```python
from build123d import *

# Parameters (mm, degrees)
SKETCH1_W              = 100
SKETCH1_H              = 100
BOSS_EXTRUDE1_DEPTH    = 10
M12_TAPPED_HOLE1_D     = 10.2
M12_TAPPED_HOLE1_DEPTH = 29.25
M12_TAPPED_HOLE1_TIP   = 3.064389157


with BuildPart() as part:
    # Sketch1 → Boss-Extrude1 (new body)
    with BuildSketch(Plane.XY):
        Rectangle(SKETCH1_W, SKETCH1_H)
    extrude(amount=BOSS_EXTRUDE1_DEPTH)

    # M12 Tapped Hole1
    with Locations(Plane.XY.offset(10)):
        with Locations((0, 30), (0, -30)):
            Hole(M12_TAPPED_HOLE1_D / 2, depth=M12_TAPPED_HOLE1_DEPTH)
            with Locations((0, 0, -(M12_TAPPED_HOLE1_DEPTH + M12_TAPPED_HOLE1_TIP / 2))):  # 118° drill point
                Cone(0, M12_TAPPED_HOLE1_D / 2, M12_TAPPED_HOLE1_TIP, mode=Mode.SUBTRACT)


solid = part.part
```
The model under review builds one solid part; all positions refer to its coordinate system, in mm. Round coordinates to 2 decimals unless told otherwise and drop trailing zeros. Write each loop counter-clockwise with the first axis right and the second up, starting at its lowest first coordinate (ties: lowest second). Pieces come first, ordered by that corner, then holes. Notation, with made-up numbers: (-30, 50) - (-24, 50) arc R8 cw to (-24, 55) - close; hole circle Ø4 at (55, -1.75). An arc over 180 degrees is marked (long way). One line per question, with ' | ' between items.
Item 1: Add section A-A, the plane y = -30. Give the boundary of the cut face in (x, z).
Resolved:
outline: (-50, 0) - (-5.1, 0) - (-5.1, 10) - (-50, 10) - close; (5.1, 0) - (50, 0) - (50, 10) - (5.1, 10) - close
Item 2: Add section C-C, the plane z = 5. Give the boundary of the cut face in (x, y).
Resolved:
outline: (-50, -50) - (50, -50) - (50, 50) - (-50, 50) - close; hole circle Ø10.2 at (0, -30); hole circle Ø10.2 at (0, 30)
Item 3: The part is to be moulded in two halves that separate along Y. For faces 1 (the face through (1, 25, 5)), 2 (the face through (-50, -1, 5)), 3 (the face through (-1, -50, 5)), say which applies: pulls with the +Y half, pulls with the -Y half, needs draft (parallel to the pull), parting line crosses it, or undercut.
Resolved:
face 1: undercut | face 2: needs draft | face 3: pulls with the -Y half
Item 4: To check wall thickness, follow probe 1 along Y at (x, z) = (0, 5.5); probe 2 along X at (y, z) = (32, 4.75); probe 3 along X at (y, z) = (-34, 7.75). State the ranges of each line that lie inside material, in increasing order.
Resolved:
probe 1: y = -50 to -35.1, -24.9 to 24.9, 35.1 to 50 | probe 2: x = -50 to -4.69, 4.69 to 50 | probe 3: x = -50 to -3.16, 3.16 to 50
Item 5: Add section B-B, the plane x = 0. Give the boundary of the cut face in (y, z).
Resolved:
outline: (-50, 0) - (-35.1, 0) - (-35.1, 10) - (-50, 10) - close; (-24.9, 0) - (24.9, 0) - (24.9, 10) - (-24.9, 10) - close; (35.1, 0) - (50, 0) - (50, 10) - (35.1, 10) - close
